For this review, take the finished solid that the model builds, in its own axes (mm). A direction names the side the tool comes from. Round coordinates to 2 decimals unless told otherwise and drop trailing zeros. Order: outer loops, then holes, each group sorted by start corner. A loop starts at its lowest first (then second) coordinate and runs counter-clockwise, first axis right, second up. Notation, with made-up numbers: (87, 60) -> (94, 60) arc R22 cw to (94, 87) -> close; hole circle Ø2 at (12, -40). An arc over 180 degrees is marked (long way). Use a Markdown table: item, result. Add a question column.
1) Draft analysis for pull direction Z (two halves, no side actions). For faces 4 (the face through (30, 143.4, 77.84)), 5 (the face through (37.1, 62.43, 150.57)), 6 (the face through (29.21, 195.178, 101.517)), 7 (the face through (14, -186, -119)), state which applies: pulls with the +Z half, pulls with the -Z half, needs draft (parallel to the pull), parting line crosses it, or undercut.
2) Wall thickness on line 1 along Y through (x, z) = (36, 0); line 2 along Z through (x, y) = (40, 79); line 3 along Z through (x, y) = (36, -3.5): over which ranges is each line inside the solid? List them lowest first. Write a range as [from, to].
3) Machinability: for faces 1 (the face through (7.098, -68.335, 216.994)), 2 (the face through (14, -142, -55)), 3 (the face through (30, 134, 134)), which of the approach directions +Z, -Z, +X, -X, +Y, -Y give a long, thin tool a straight path to every point of the face, cutting with its end or side? Answer none if there is none.
4) Consider section C-C (x = 22.5). State the section outline as (y, z) points, plus the area to 3 significant figures.
5) Clearance check with flat-ended pins moving along their axes: P1, Ø8, axis at x = 25, y = -43, coming from the -Z side; P2, Ø8, axis at x = 23, y = 180, coming from the +Z side; P3, Ø1, axis at x = 17.5, y = 131, coming from the +Z side. State where each tip first meets the part, or that it passes through.
```python
from build123d import *

# Parameters (mm, degrees)
FILLET1_R = 10


with BuildPart() as part:
    # Sketch1 → Revolve1 (revolve)
    with BuildSketch(Plane(origin=(0, 0, 0), x_dir=(1, 0, 0), z_dir=(0, 1, 0)), mode=Mode.PRIVATE) as revolve1_sk:
        Polygon((0, 200), (0, 227.5), (14, 227.5), (14, 220), (44, 220), (44, 203), (30, 203), (30, 189), (44, 189), (44, 177), (30, 177), (30, 163), (44, 163), (44, 151), (14, 151), (14, 200), align=None)
    revolve(revolve1_sk.sketch.rotate(Axis((0, 0, 0), (1, 0, 0)), 180), axis=Axis((0, 0, 0), (1, 0, 0)))

    # Fillet1
    fillet1_edges = [part.edges().sort_by_distance(p)[0] for p in [
        (14, 0, -200),
    ]]
    fillet(fillet1_edges, radius=FILLET1_R)


solid = part.part
```
Results list:
| question | item | result |
|---|---|---|
| 1 | face 4 | undercut |
| 1 | face 5 | undercut |
| 1 | face 6 | parting line crosses it |
| 1 | face 7 | needs draft |
| 2 | line 1 | [-220, -203], [-189, -177], [-163, -151], [151, 163], [177, 189], [203, 220] |
| 2 | line 2 | [-205.33, -187], [-171.7, -158.39], [-142.58, -128.69], [128.69, 142.58], [158.39, 171.7], [187, 205.33] |
| 2 | line 3 | [-219.97, -202.97], [-188.97, -176.97], [-162.96, -150.96], [150.96, 162.96], [176.97, 188.97], [202.97, 219.97] |
| 3 | face 1 | +X, -X |
| 3 | face 2 | -X |
| 3 | face 3 | +X |
| 4 | outline | circle Ø440 at (0, 0); hole circle Ø302 at (0, 0) |
| 4 | area | 80,400 mm2 |
| 5 | P1 | z = -216.52 |
| 5 | P2 | z = 132 |
| 5 | P3 | z = 177.12 |
